Geometry check sheet. Reference: the model listing, model coordinates, mm. Round coordinates to 2 decimals unless told otherwise and drop trailing zeros. Loops run counter-clockwise (first coordinate to the right, second up) from the corner with the lowest first, then second, coordinate; pieces in that order, holes last.
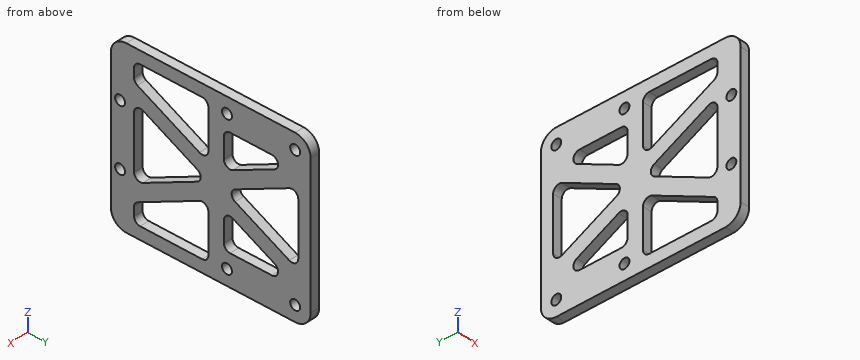
```python
from build123d import *

# Parameters (mm, degrees)
SKETCH_2_W          = 55
SKETCH_2_H          = 64.5
EXTRUDE_1_DEPTH     = 3
SKETCH_3_R          = 1.6
CUT_EXTRUDE_1_DEPTH = 3
FILLET_1_R          = 5
CUT_EXTRUDE_2_DEPTH = 3
FILLET_2_R          = 2


with BuildPart() as part:
    # 草图2 → 凸台-拉伸1 (new body)
    with BuildSketch(Plane(origin=(0, 0, 0), x_dir=(0, 0, -1), z_dir=(1, 0, 0))):
        with Locations((27.5, 32.25)):
            Rectangle(SKETCH_2_W, SKETCH_2_H)
    extrude(amount=EXTRUDE_1_DEPTH)

    # 草图3 → 切除-拉伸1 (cut)
    with BuildSketch(Plane.ZY):
        with Locations((-5, 59.5)):
            Circle(SKETCH_3_R)
        with Locations((-5, 37.5)):
            Circle(SKETCH_3_R)
        with Locations((-50, 59.5)):
            Circle(SKETCH_3_R)
        with Locations((-50, 37.5)):
            Circle(SKETCH_3_R)
        with Locations((-37.5, 3)):
            Circle(SKETCH_3_R)
        with Locations((-17.5, 3)):
            Circle(SKETCH_3_R)
    extrude(amount=-CUT_EXTRUDE_1_DEPTH, mode=Mode.SUBTRACT)

    # 圆角1
    fillet_1_edges = [part.edges().sort_by_distance(p)[0] for p in [
        (1.5, 64.5, 0),
        (1.5, 64.5, -55),
        (1.5, 0, -55),
        (1.5, 0, 0),
    ]]
    fillet(fillet_1_edges, radius=FILLET_1_R)

    # 草图4 → 切除-拉伸2 (cut)
    with BuildSketch(Plane.ZY):
        Polygon((-39.417495765, 60.5), (-27.5, 36.5), (-15.582504235, 60.5), align=None)
        Polygon((-45, 60.5), (-45, 36.5), (-33.082504235, 36.5), align=None)
        Polygon((-21.917495765, 36.5), (-10, 60.5), (-10, 36.5), align=None)
        Polygon((-10, 31.5), (-21.917495765, 31.5), (-10, 7.5), (-4, 7.5), (-4, 31.5), align=None)
        Polygon((-39.417495765, 7.5), (-27.5, 31.5), (-15.582504235, 7.5), align=None)
        Polygon((-45, 31.5), (-33.082504235, 31.5), (-45, 7.5), (-51, 7.5), (-51, 31.5), align=None)
    extrude(amount=-CUT_EXTRUDE_2_DEPTH, mode=Mode.SUBTRACT)

    # 圆角2
    fillet_2_edges = [part.edges().sort_by_distance(p)[0] for p in [
        (1.5, 60.5, -45),
        (1.5, 36.5, -33.082504235),
        (1.5, 36.5, -45),
        (1.5, 60.5, -39.417495765),
        (1.5, 60.5, -15.582504235),
        (1.5, 36.5, -27.5),
        (1.5, 31.5, -27.5),
        (1.5, 7.5, -15.582504235),
        (1.5, 7.5, -39.417495765),
        (1.5, 31.5, -4),
        (1.5, 7.5, -4),
        (1.5, 7.5, -10),
        (1.5, 31.5, -21.917495765),
        (1.5, 7.5, -51),
        (1.5, 31.5, -51),
        (1.5, 31.5, -33.082504235),
        (1.5, 7.5, -45),
        (1.5, 36.5, -10),
        (1.5, 36.5, -21.917495765),
        (1.5, 60.5, -10),
    ]]
    fillet(fillet_2_edges, radius=FILLET_2_R)


solid = part.part
```
1) Sectioned sample at A-A, the plane z = -33. Record the cut outline in (x, y).
Report:
outline: (0, 0) - (3, 0) - (3, 7.5) - (0, 7.5) - close; (0, 20.42) - (3, 20.42) - (3, 47.58) - (0, 47.58) - close; (0, 60.5) - (3, 60.5) - (3, 64.5) - (0, 64.5) - close
2) Sectioned sample at B-B, the plane y = 37.5. Record the cut outline in (x, z), then the cut area to 3 significant figures.
Report:
outline: (0, -55) - (3, -55) - (3, -51.6) - (0, -51.6) - close; (0, -48.4) - (3, -48.4) - (3, -44.73) - (0, -44.73) - close; (0, -34.58) - (3, -34.58) - (3, -20.42) - (0, -20.42) - close; (0, -10.27) - (3, -10.27) - (3, -6.6) - (0, -6.6) - close; (0, -3.4) - (3, -3.4) - (3, 0) - (0, 0) - close
area: 84.9 mm2
3) Sectioned sample at D-D, the plane y = 47.5. Record the cut outline in (x, z).
Report:
outline: (0, -55) - (3, -55) - (3, -45) - (0, -45) - close; (0, -38.54) - (3, -38.54) - (3, -32.96) - (0, -32.96) - close; (0, -22.04) - (3, -22.04) - (3, -16.46) - (0, -16.46) - close; (0, -10) - (3, -10) - (3, 0) - (0, 0) - close
4) Sectioned sample at C-C, the plane x = 1.3. State how many separate pieces and enclosed holes the cut face has, then the cut area to 3 significant figures.
Report:
separate pieces: 1
enclosed holes: 12
area: 2,100 mm2
5) Scan lines: line 1 along Y through (x, z) = (2.4, -48); line 2 along Z through (x, y) = (0.35, 24); line 3 along Y through (x, z) = (2.55, -49.5). Record each from-to range of solid material in increasing order.
Report:
line 1: y = 0 to 7.5, 31.5 to 64.5
line 2: z = -55 to -51, -36.81 to -31.22, -23.78 to -18.19, -4 to 0
line 3: y = 0 to 7.56, 31.44 to 35.98, 39.02 to 57.98, 61.02 to 64.5
